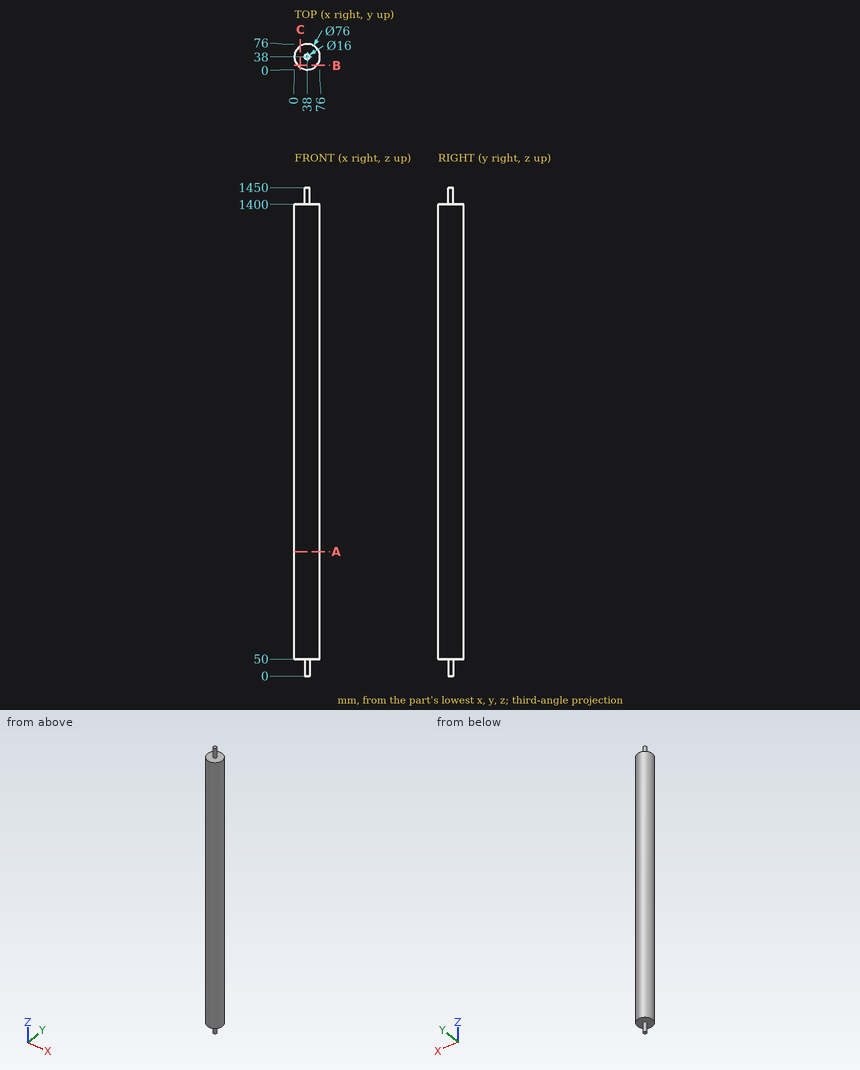
Verification items for this drawing (mm, ordinates from the low corner). Coordinates: 2 decimals unless noted, no trailing zeros. Write each loop counter-clockwise with the first axis right and the second up, starting at its lowest first coordinate (ties: lowest second). Pieces come first, ordered by that corner, then holes. Notation, with made-up numbers: M -8,83.25 L 50,83.25 A26 cw 50,103.25 Z; hole C 85.5,-3.5 d7. An arc over 180 degrees is marked long. Use one line per item in the form item = value. Start each with the question number.
1) Thickness scan on probe 1 along Z at (x, y) = (4, 31); probe 2 along X at (y, z) = (37.5, 898.5); probe 3 along Y at (x, z) = (33.5, 1030). Record the ranges inside material, lowest first. Write a range as from..to.
2) Go/stop test with flat-tipped pins: pin 1 Ø1.5 at (x, z) = (8.5, 529) entering from -Y; pin 2 Ø10 at (y, z) = (56, 653.5) entering from -X; pin 3 Ø12 at (y, z) = (53.5, 429) entering from +X. Record where each tip stops, or that it passes through.
3) Section check B-B on y = 12.5. Enter the section's corners in (x, z).
4) Section check A-A on z = 369. Enter the section's corners in (x, y).
5) Section check C-C on x = 17.5. Enter the section's corners in (y, z).
Responses:
q1.probe_1 = 50..1400
q1.probe_2 = 0..76
q1.probe_3 = 0.27..75.73
q2.pin_1 = 13.15
q2.pin_2 = 2.29
q2.pin_3 = 74.79
q3.outline = M 9.83,50 L 66.17,50 L 66.17,1400 L 9.83,1400 Z
q4.outline = C 38,38 d76
q5.outline = M 6,50 L 70,50 L 70,1400 L 6,1400 Z
